Can you work these out from the drawing? Everything is in mm from the part's minimum corner. A direction names the side the tool comes from. Coordinates: 2 decimals unless noted, no trailing zeros. Order: outer loops, then holes, each group sorted by start corner. A loop starts at its lowest first (then second) coordinate and runs counter-clockwise, first axis right, second up. Notation, with made-up numbers: (57, 58.25) -> (93, 58.25) arc R31 ccw to (93, 90.25) -> close; hole circle Ø2 at (11.5, 39.25). An arc over 180 degrees is marked (long way). Put each result on its own line as item: value. Start each with the question number.
Q1. We'd pull the mould along Y, two halves only. Please class the marked faces 3, 4, 5 and 6: +Y half, -Y half, draft (parallel to the pull), parting line (faces both ways), or undercut.
Q2. If we section it at D-D (z = 2.25): Please give me the cut outline in (x, y), and give its area (3 significant figures).
Q3. If we section it at C-C (y = 9.75): Please give me the cut outline in (x, z), and give its area (3 significant figures).
Q4. If we section it at B-B (x = 3.25): Please give me the cut outline in (y, z).
Q5. For the marked faces 1 and 2, which set-ups out of +Z, -Z, +X, -X, +Y, -Y let a thin tool reach every point of the face, with its end or its side?
Q6. Will these pins go through, and if not, where does the flat tip stop? pin 1 (1 mm diameter, centred on x = 3, y = 10, fed in from -Z); pin 2 (2 mm diameter, centred on y = 8.5, z = 3, fed in from +X); pin 3 (2 mm diameter, centred on x = 5.5, y = 5, fed in from -Z).
Q7. Please list where these lines run through material, in increasing order: line 1 along X through (y, z) = (7.5, 7); line 2 along Z through (x, y) = (8.5, 5.25); line 3 along Z through (x, y) = (4.5, 5.75).
Q8. If we section it at A-A (z = 7): Please give me the cut outline in (x, y), and give its area (3 significant figures).
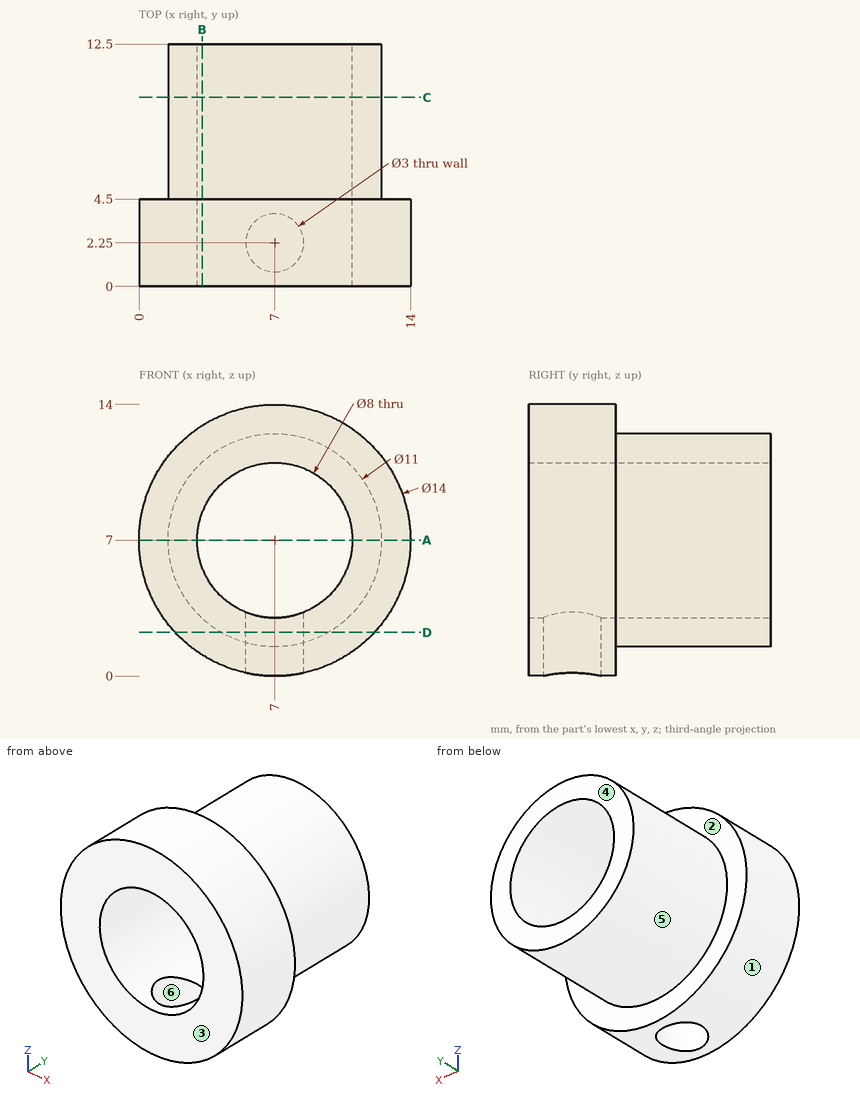
The answers:
1. face 3: -Y half
1. face 4: +Y half
1. face 5: draft
1. face 6: undercut
2. outline: (1.86, 0) -> (12.14, 0) -> (12.14, 4.5) -> (9.77, 4.5) -> (9.77, 12.5) -> (4.23, 12.5) -> (4.23, 4.5) -> (1.86, 4.5) -> close; hole circle Ø3 at (7, 2.25)
2. area: 83.6 mm^2
3. outline: circle Ø11 at (7, 7); hole circle Ø8 at (7, 7)
3. area: 44.8 mm^2
4. outline: (0, 1.09) -> (4.5, 1.09) -> (4.5, 2.98) -> (12.5, 2.98) -> (12.5, 5.61) -> (0, 5.61) -> close; (0, 8.39) -> (12.5, 8.39) -> (12.5, 11.02) -> (4.5, 11.02) -> (4.5, 12.91) -> (0, 12.91) -> close
5. face 1: +Y, -Y
5. face 2: +Y
6. pin 1: z = 2.76
6. pin 2: x = 11.61
6. pin 3: z = 0.03
7. line 1: 1.5 to 3, 11 to 12.5
7. line 2: 1.71 to 3.29, 10.71 to 12.29
7. line 3: 2.1 to 3.88, 10.12 to 11.9
8. outline: (0, 0) -> (3, 0) -> (3, 12.5) -> (1.5, 12.5) -> (1.5, 4.5) -> (0, 4.5) -> close; (11, 0) -> (14, 0) -> (14, 4.5) -> (12.5, 4.5) -> (12.5, 12.5) -> (11, 12.5) -> close
8. area: 51.0 mm^2
